from build123d import *

# Parameters (mm, degrees)
SKETCH_1_W                = 300
SKETCH_1_H                = 80
EXTRUDE_1_DEPTH           = 20
CHAMFER_1_SIZE            = 3
HOLE_WIZARD_1_D           = 15.5
HOLE_WIZARD_1_DEPTH       = 25
HOLE_WIZARD_1_CBORE_D     = 24
HOLE_WIZARD_1_CBORE_DEPTH = 15
HOLE_WIZARD_1_TIP         = 4.656669797
HOLE_WIZARD_0_D           = 6.6
HOLE_WIZARD_0_DEPTH       = 25
HOLE_WIZARD_0_CBORE_D     = 11
HOLE_WIZARD_0_CBORE_DEPTH = 6.8
HOLE_WIZARD_0_TIP         = 1.982840043
SKETCH_6_R                = 10
SKETCH_6_R_2              = 8.1
CUT_EXTRUDE_1_DEPTH       = 2
HOLE_WIZARD_M5_1_D        = 4.2
HOLE_WIZARD_M5_2_D        = 4.2
HOLE_WIZARD_M5_2_DEPTH    = 12.4
HOLE_WIZARD_M5_2_TIP      = 1.2618073


with BuildPart() as part:
    # 草图1 → 凸台-拉伸1 (new body)
    with BuildSketch(Plane(origin=(0, 0, 0), x_dir=(1, 0, 0), z_dir=(0, 1, 0))):
        Rectangle(SKETCH_1_W, SKETCH_1_H)
    extrude(amount=EXTRUDE_1_DEPTH)

    # 倒角1
    chamfer_1_edges = [part.edges().sort_by_distance(p)[0] for p in [
        (150, 10, 40),
        (-150, 10, 40),
        (-150, 10, -40),
        (150, 10, -40),
    ]]
    chamfer(chamfer_1_edges, length=CHAMFER_1_SIZE)

    # 打孔尺寸(%根据)内六角圆柱头螺钉的类型1
    with Locations(Plane(origin=(0, 20, 0), x_dir=(1, 0, 0), z_dir=(0, 1, 0))):
        with Locations((-25, 0)):
            CounterBoreHole(HOLE_WIZARD_1_D / 2, HOLE_WIZARD_1_CBORE_D / 2, HOLE_WIZARD_1_CBORE_DEPTH, depth=HOLE_WIZARD_1_DEPTH)
            with Locations((0, 0, -(HOLE_WIZARD_1_DEPTH + HOLE_WIZARD_1_TIP / 2))):  # 118° drill point
                Cone(0, HOLE_WIZARD_1_D / 2, HOLE_WIZARD_1_TIP, mode=Mode.SUBTRACT)

    # 打孔尺寸(%根据)内六角圆柱头螺钉的类型0
    with Locations(Plane(origin=(0, 20, 0), x_dir=(1, 0, 0), z_dir=(0, 1, 0))):
        with Locations((30, 30), (-80, 30), (30, -30), (-80, -30)):
            CounterBoreHole(HOLE_WIZARD_0_D / 2, HOLE_WIZARD_0_CBORE_D / 2, HOLE_WIZARD_0_CBORE_DEPTH, depth=HOLE_WIZARD_0_DEPTH)
            with Locations((0, 0, -(HOLE_WIZARD_0_DEPTH + HOLE_WIZARD_0_TIP / 2))):  # 118° drill point
                Cone(0, HOLE_WIZARD_0_D / 2, HOLE_WIZARD_0_TIP, mode=Mode.SUBTRACT)

    # 草图6 → 切除-拉伸1 (cut)
    with BuildSketch(Plane.XZ):
        with Locations(Location((-25, 0, 0), (0, 0, 270))):
            Circle(SKETCH_6_R)
        with Locations(Location((30, -30, 0), (0, 0, 270))):
            Circle(SKETCH_6_R_2)
        with Locations(Location((-80, -30, 0), (0, 0, 270))):
            Circle(SKETCH_6_R_2)
        with Locations(Location((30, 30, 0), (0, 0, 270))):
            Circle(SKETCH_6_R_2)
        with Locations(Location((-80, 30, 0), (0, 0, 270))):
            Circle(SKETCH_6_R_2)
    extrude(amount=-CUT_EXTRUDE_1_DEPTH, mode=Mode.SUBTRACT)

    # M5 螺纹孔1 (through all)
    with Locations(Plane(origin=(0, 0, 0), x_dir=(-1, 0, 0), z_dir=(0, -1, 0))):
        with Locations((-96, -15), (-96, 15), (4, -15), (4, 15), (104, -15), (104, 15)):
            Hole(HOLE_WIZARD_M5_1_D / 2)

    # M5 螺纹孔2
    with Locations(Plane(origin=(0, 0, -40), x_dir=(-1, 0, 0), z_dir=(0, 0, -1))):
        with Locations((-142, 10), (-130, 10)):
            Hole(HOLE_WIZARD_M5_2_D / 2, depth=HOLE_WIZARD_M5_2_DEPTH)
            with Locations((0, 0, -(HOLE_WIZARD_M5_2_DEPTH + HOLE_WIZARD_M5_2_TIP / 2))):  # 118° drill point
                Cone(0, HOLE_WIZARD_M5_2_D / 2, HOLE_WIZARD_M5_2_TIP, mode=Mode.SUBTRACT)


solid = part.part
Geometry check sheet. Reference: the model listing, model coordinates, mm. A direction names the side the tool comes from. Give positions to 0.01 mm unless a question says otherwise; leave off trailing zeros. Loops run counter-clockwise (first coordinate to the right, second up) from the corner with the lowest first, then second, coordinate; pieces in that order, holes last. Notation, with made-up numbers: (85.25, 25.5) -> (97.25, 25.5) arc R21 cw to (97.25, 42.5) -> close; hole circle Ø5 at (41, 64.25). An arc over 180 degrees is marked (long way). Answer in a Markdown table with one row per item. Add a question column.
1) Cross-section at C-C on z = 4. Record the boundary of the cut face in (x, y), and give its area (3 significant figures).
2) Cross-section at B-B on z = 30. Record the boundary of the cut face in (x, y).
3) Material ranges on probe 1 along Z at (x, y) = (96, 12); probe 2 along X at (y, z) = (10, -35); probe 3 along X at (y, z) = (5, 15), recorded low to high. Write a range as from..to.
4) Set-up check for faces 1 (the face through (-83.5, 2, -29.9)), 2 (the face through (26.85, 7.52, 29.01)), 3 (the face through (-76, 13.2, 30)): record each of +Z, -Z, +X, -X, +Y, -Y from which the full face is reachable in a straight line by a thin tool's end or side.
5) Gauge pin test, flat ends, axial feed: P1, Ø8, axis at x = 33.5, z = -28, coming from the -Y side; P2, Ø10.5, axis at x = -80, z = -30, coming from the +Y side. Record the tip position at first contact, or that the pin passes through.
6) Cross-section at A-A on y = 16. State how many separate pieces and enclosed holes the cut face has, and give its area (3 significant figures).
7) Draft check along Z on faces 4 (the face through (-2, 10, -40)), 5 (the face through (-150, 10, 1)), 6 (the face through (-32.4, 3.5, -2.3)), 7 (the face through (-76, 13.2, -30)). Enter one of: pulls with the +Z half, pulls with the -Z half, needs draft (parallel to the pull), parting line crosses it, or undercut.
Outcome:
| question | item | result |
|---|---|---|
| 1 | outline | (-150, 0) -> (-34.17, 0) -> (-34.17, 2) -> (-31.64, 2) -> (-31.64, 5) -> (-36.31, 5) -> (-36.31, 20) -> (-150, 20) -> close; (-18.36, 2) -> (-15.83, 2) -> (-15.83, 0) -> (150, 0) -> (150, 20) -> (-13.69, 20) -> (-13.69, 5) -> (-18.36, 5) -> close |
| 1 | area | 5,580 mm^2 |
| 2 | outline | (-150, 0) -> (-88.1, 0) -> (-88.1, 2) -> (-83.3, 2) -> (-83.3, 13.2) -> (-85.5, 13.2) -> (-85.5, 20) -> (-150, 20) -> close; (-76.7, 2) -> (-71.9, 2) -> (-71.9, 0) -> (21.9, 0) -> (21.9, 2) -> (26.7, 2) -> (26.7, 13.2) -> (24.5, 13.2) -> (24.5, 20) -> (-74.5, 20) -> (-74.5, 13.2) -> (-76.7, 13.2) -> close; (33.3, 2) -> (38.1, 2) -> (38.1, 0) -> (150, 0) -> (150, 20) -> (35.5, 20) -> (35.5, 13.2) -> (33.3, 13.2) -> close |
| 3 | probe 1 | z = -40..-17.1, -12.9..12.9, 17.1..40 |
| 3 | probe 2 | x = -150..127.9, 132.1..139.9, 144.1..150 |
| 3 | probe 3 | x = -150..-106.1, -101.9..-6.1, -1.9..93.9, 98.1..150 |
| 4 | face 1 | -Y |
| 4 | face 2 | +Y, -Y |
| 4 | face 3 | +Y |
| 5 | P1 | stops at y = 2 |
| 5 | P2 | stops at y = 13.2 |
| 6 | separate pieces | 1 |
| 6 | enclosed holes | 11 |
| 6 | area | 23,100 mm^2 |
| 7 | face 4 | pulls with the -Z half |
| 7 | face 5 | needs draft |
| 7 | face 6 | undercut |
| 7 | face 7 | undercut |
